Here's the drawing with two shaded views (mm, measured from the low corner). I have some questions. Round coordinates to 2 decimals unless told otherwise and drop trailing zeros. Loops run counter-clockwise (first coordinate to the right, second up) from the corner with the lowest first, then second, coordinate; pieces in that order, holes last.
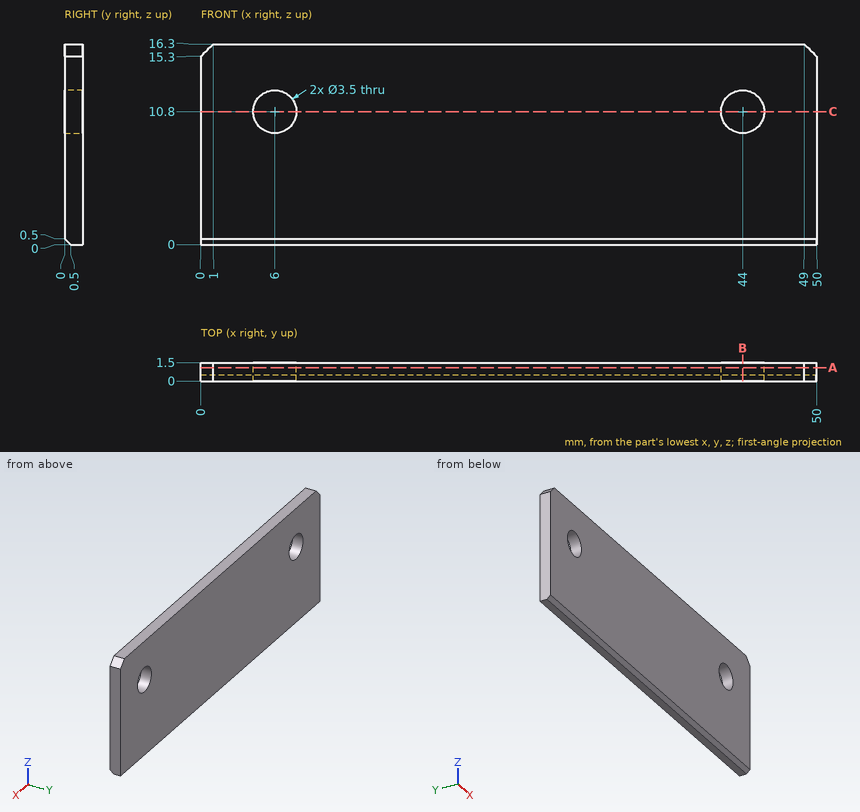
Item 1: If we section it at C-C, the plane z = 10.8: Please give me the cut outline in (x, y), then the cut area to 3 significant figures.
Results list:
outline: (0, 0) - (4.25, 0) - (4.25, 1.5) - (0, 1.5) - close; (7.75, 0) - (42.25, 0) - (42.25, 1.5) - (7.75, 1.5) - close; (45.75, 0) - (50, 0) - (50, 1.5) - (45.75, 1.5) - close
area: 64.5 mm2
Item 2: If we section it at B-B, the plane x = 44: Please give me the cut outline in (y, z).
Results list:
outline: (0, 0.5) - (0.5, 0) - (1.5, 0) - (1.5, 9.05) - (0, 9.05) - close; (0, 12.55) - (1.5, 12.55) - (1.5, 16.3) - (0, 16.3) - close
Item 3: If we section it at A-A, the plane y = 1.1: Please give me the cut outline in (x, z).
Results list:
outline: (0, 0) - (50, 0) - (50, 15.3) - (49, 16.3) - (1, 16.3) - (0, 15.3) - close; hole circle Ø3.5 at (6, 10.8); hole circle Ø3.5 at (44, 10.8)
Item 4: Will this pin go through, and if not, where does the flat tip stop? pin 1 (4.5 mm diameter, centred on x = 44, z = 10.8, fed in from -Y).
Results list:
pin 1: stops at y = 0
Item 5: If I drill on line 1 along X through (y, z) = (0.4, 10.8); line 2 along Z through (x, y) = (45, 1.45); line 3 along Z through (x, y) = (17.5, 0.2), over which ranges is the centre line in solid material (lowest first)?
Results list:
line 1: x = 0 to 4.25, 7.75 to 42.25, 45.75 to 50
line 2: z = 0 to 9.36, 12.24 to 16.3
line 3: z = 0.3 to 16.3
